Verification items for this drawing (mm, ordinates from the low corner). A direction names the side the tool comes from. Coordinates: 2 decimals unless noted, no trailing zeros. Loops run counter-clockwise (first coordinate to the right, second up) from the corner with the lowest first, then second, coordinate; pieces in that order, holes last. Notation, with made-up numbers: (34, -37.75) -> (89, -37.75) arc R16 cw to (89, -29.75) -> close; hole circle Ø10 at (-17.75, 70.25). An arc over 180 degrees is marked (long way). Write item = value, one per line.
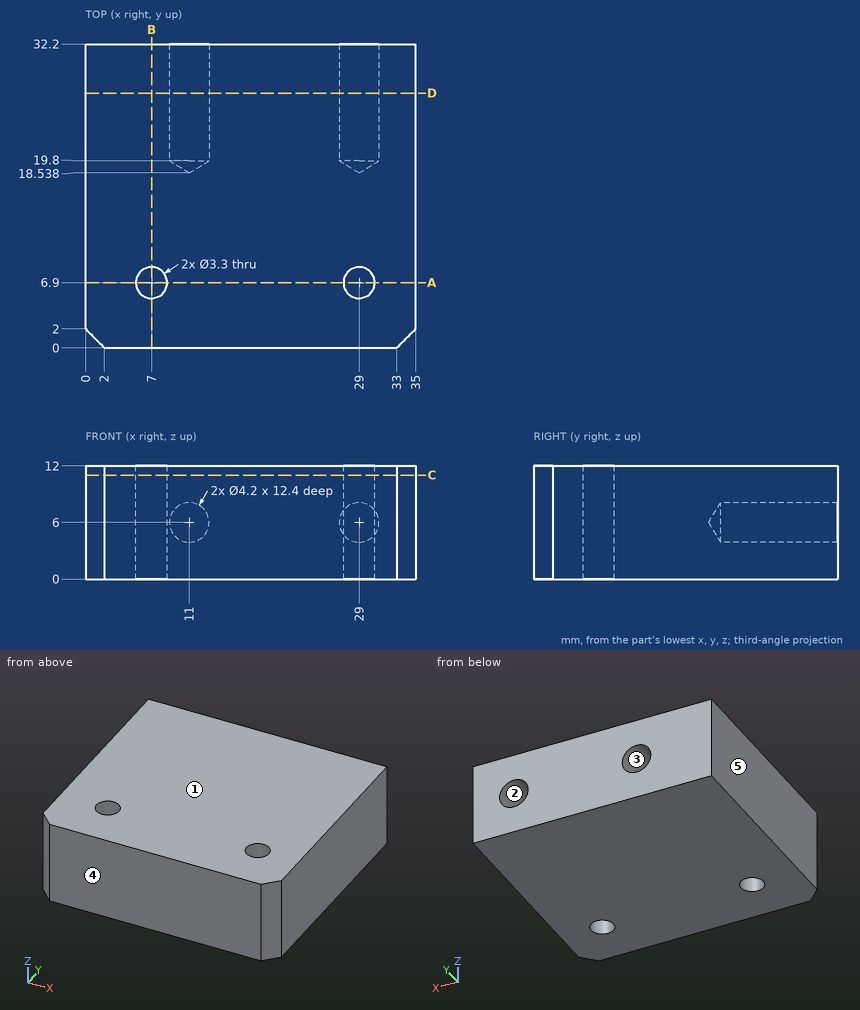
1) Sectioned sample at C-C, the plane z = 11. Record the cut outline in (x, y).
Ans:
outline = (0, 2) -> (2, 0) -> (33, 0) -> (35, 2) -> (35, 32.2) -> (0, 32.2) -> close; hole circle Ø3.3 at (7, 6.9); hole circle Ø3.3 at (29, 6.9)
2) Release check for a two-part mould opening along X. For the marked faces 3, 4 and 5 record: pulls with the +X half, pulls with the -X half, needs draft (parallel to the pull), parting line crosses it, or undercut.
Ans:
face_3 = undercut
face_4 = needs draft
face_5 = pulls with the -X half
3) Material ranges on line 1 (X direction, y = 26.25, z = 6); line 2 (Z direction, x = 29, y = 24.75); line 3 (X direction, y = 5.5, z = 11.25), recorded low to high.
Ans:
line_1 = 0 to 8.9, 13.1 to 26.9, 31.1 to 35
line_2 = 0 to 3.9, 8.1 to 12
line_3 = 0 to 6.13, 7.87 to 28.13, 29.87 to 35
4) Sectioned sample at B-B, the plane x = 7. Record the cut outline in (y, z), plus the area to 3 significant figures.
Ans:
outline = (0, 0) -> (5.25, 0) -> (5.25, 12) -> (0, 12) -> close; (8.55, 0) -> (32.2, 0) -> (32.2, 12) -> (8.55, 12) -> close
area = 347 mm2
5) Tool access check on the marked faces 1 and 2. Record the directions out of +Z, -Z, +X, -X, +Y, -Y that give a thin tool (end or side, any length) a straight path to the whole face; none if there is none.
Ans:
face_1 = +Z, +X, -X, +Y, -Y
face_2 = +Y
6) Sectioned sample at D-D, the plane y = 27. Record the cut outline in (x, z), plus the area to 3 significant figures.
Ans:
outline = (0, 0) -> (35, 0) -> (35, 12) -> (0, 12) -> close; hole circle Ø4.2 at (11, 6); hole circle Ø4.2 at (29, 6)
area = 392 mm2
7) Sectioned sample at A-A, the plane y = 6.9. Record the cut outline in (x, z), plus the area to 3 significant figures.
Ans:
outline = (0, 0) -> (5.35, 0) -> (5.35, 12) -> (0, 12) -> close; (8.65, 0) -> (27.35, 0) -> (27.35, 12) -> (8.65, 12) -> close; (30.65, 0) -> (35, 0) -> (35, 12) -> (30.65, 12) -> close
area = 341 mm2
8) Depth check by flat-ended pin: pin 1 Ø4 at (x, z) = (11, 6) entering from +Y. Enter the tip coordinate at first touch or a pass-through.
Ans:
pin_1 = 19.74
